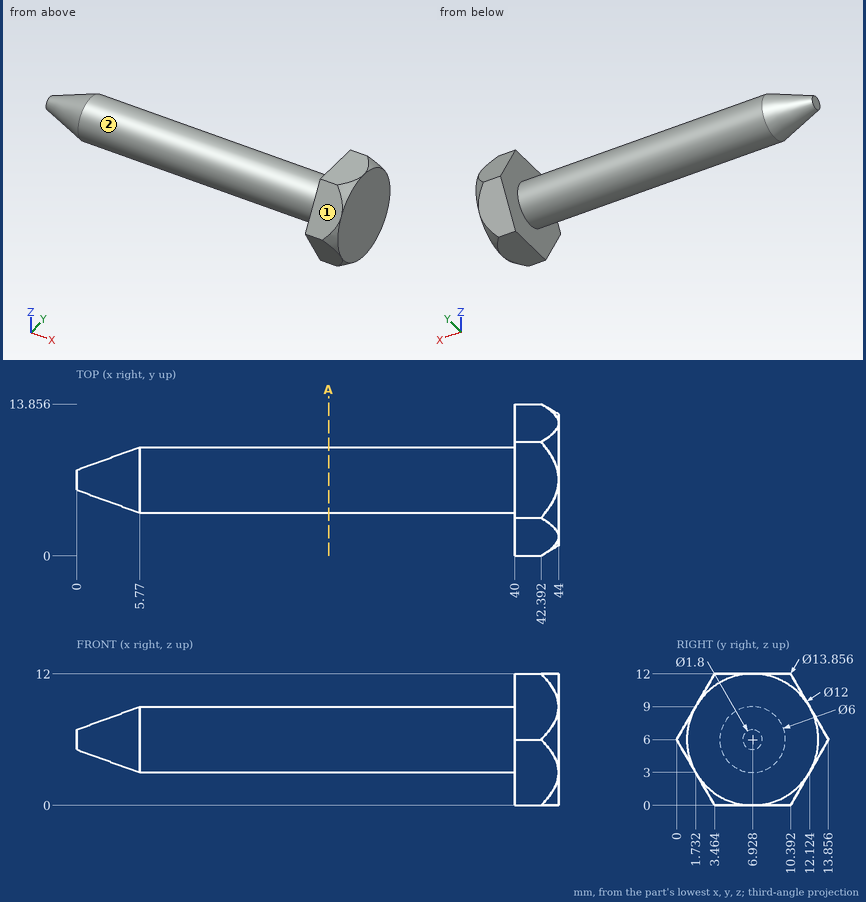
Geometry check sheet. Reference: drawing and pictorial views, mm from the part's lowest x, y, z. A direction names the side the tool comes from. Give positions to 0.01 mm unless a question says otherwise; leave off trailing zeros. Write each loop counter-clockwise with the first axis right and the second up, starting at its lowest first coordinate (ties: lowest second). Pieces come first, ordered by that corner, then holes.
Item 1: Cross-section at A-A (x = 23). Enter the section's corners in (y, z), and give its area (3 significant figures).
Item 2: Access from +Z, -Z, +X, -X, +Y, -Y to the whole of each face (thin tool, end or side, straight path). Record for the marked faces 1 and 2.
Item 3: Scan lines: L1, parallel to Y at x = 23.5, z = 6; L2, parallel to X at y = 11.75, z = 3.25; L3, parallel to Y at x = 31, z = 8.5 (1 decimal). Record each from-to range of solid material in increasing order.
Item 4: Gauge pin test, flat ends, axial feed: pin 1 (1.5 mm diameter, centred on x = 28, y = 8.5, fed in from -Z) (1 decimal); pin 2 (4 mm diameter, centred on x = 7.5, y = 1.5, fed in from +Z); pin 3 (4 mm diameter, centred on x = 14.5, y = 11, fed in from -Z); pin 4 (1 mm diameter, centred on x = 20, z = 6.5, fed in from +Y). Record the tip position at first contact, or that the pin passes through.
Report:
1. outline: circle Ø6 at (6.93, 6)
1. area: 28.3 mm2
2. face 1: +Z, +X, -X, -Y
2. face 2: -X
3. L1: y = 3.93 to 9.93
3. L2: x = 40 to 44
3. L3: y = 5.3 to 8.6
4. pin 1: stops at z = 3.1
4. pin 2: passes through
4. pin 3: stops at z = 3.83
4. pin 4: stops at y = 9.93
